Study the drawing (mm; zero at the part's minimum x, y, z) and answer. A direction names the side the tool comes from. Coordinates: 2 decimals unless noted, no trailing zeros. Loops run counter-clockwise (first coordinate to the right, second up) from the corner with the lowest first, then second, coordinate; pieces in that order, holes last. Notation, with made-up numbers: (73.25, -6.75) - (81.25, -6.75) arc R23 cw to (81.25, 13.25) - close; hole circle Ø1 at (72, -31.75). An arc over 180 degrees is marked (long way). Put each result on its own line as item: value.
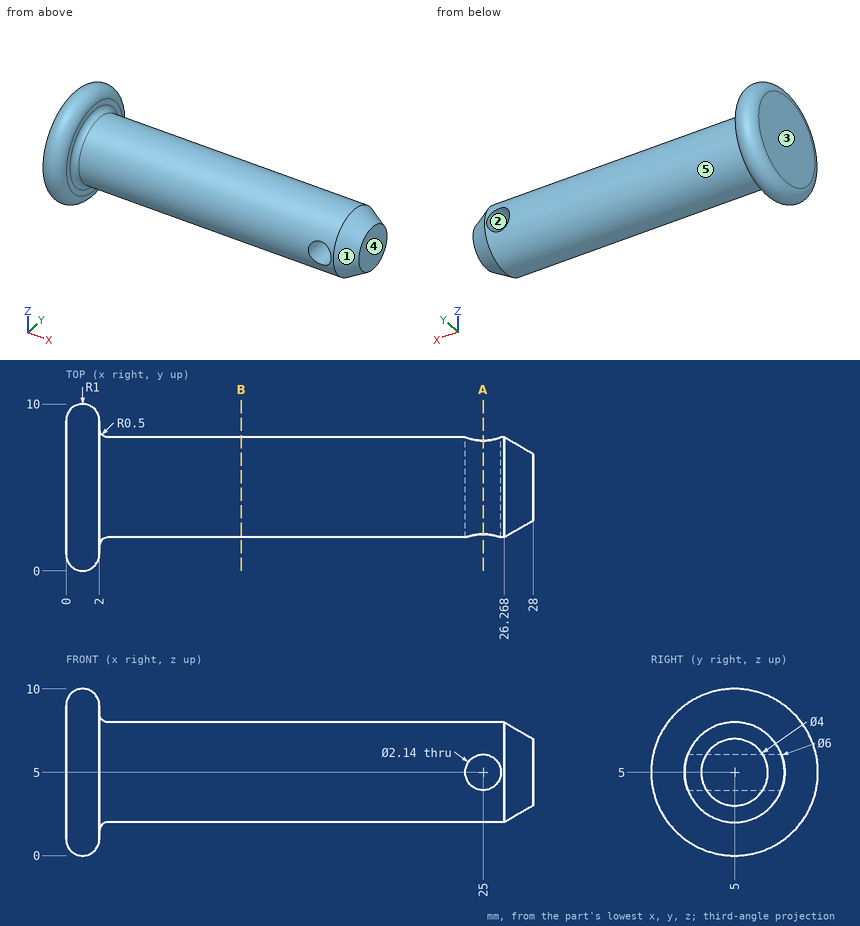
1) For a pull along X with two mould halves and no side action, classify the marked faces 1, 2 and 3 as pulls with the +X half, pulls with the -X half, needs draft (parallel to the pull), parting line crosses it, or undercut.
Found:
face 1: pulls with the +X half
face 2: undercut
face 3: pulls with the -X half
2) Each of these flat-tipped pins is pushed along its axis until it touches: pin 1 (6 mm diameter, centred on y = 7, z = 3, fed in from -X); pin 2 (1 mm diameter, centred on x = 23, y = 4.5, fed in from +Z); pin 3 (3 mm diameter, centred on x = 25, z = 5, fed in from +Y). Where does it stop, or does it pass through?
Found:
pin 1: stops at x = 0
pin 2: stops at z = 8
pin 3: stops at y = 8
3) For the marked faces 4 and 5, determine the directions among +Z, -Z, +X, -X, +Y, -Y from which every point of the face is accessible in a straight line to the end or side of a thin tool.
Found:
face 4: +Z, -Z, +X, +Y, -Y
face 5: +X
4) The part is cut by section B-B (x = 10.5). Give the vertices of the cut face in (y, z), and give its area (3 significant figures).
Found:
outline: circle Ø6 at (5, 5)
area: 28.3 mm^2
5) The part is cut by section A-A (x = 25). Give the vertices of the cut face in (y, z), and give its area (3 significant figures).
Found:
outline: (2.2, 3.93) arc R3 ccw to (7.8, 3.93) - close; (2.2, 6.07) - (7.8, 6.07) arc R3 ccw to start
area: 15.7 mm^2
6) Straight lines are drawn through the part: L1, parallel to X at y = 6.5, z = 5; L2, parallel to X at y = 7.5, z = 1.75 (3 decimals); L3, parallel to Z at x = 25, y = 6. For each, find the intervals that lie inside material, in ascending order. Write a range as [from, to].
Found:
L1: x = [0, 23.93], [26.07, 28]
L2: x = [0.005, 1.995]
L3: z = [2.17, 3.93], [6.07, 7.83]
